```python
from build123d import *

# Parameters (mm, degrees)
V_BLOCK_BODY_100_DEPTH    = 100
CENTRAL_CHANNEL_SKETCH_W  = 36
CENTRAL_CHANNEL_SKETCH_H  = 12
CENTRAL_CHANNEL_CUT_DEPTH = 166
SQUARE_POCKET_18X18_REACH = 179.739
SQUARE_START              = -32
SQUARE_POCKET_SKETCH_W    = 88
SQUARE_POCKET_SKETCH_H    = 60
ANGLED_NOTCH_CUT_REACH    = 131.46


with BuildPart() as part:
    # V-Block Profile Sketch → V-Block Body 100 (new body)
    with BuildSketch(Plane.XY):
        Polygon((-30, 43), (0, 13), (30, 43), (62, 43), (62, -43), (-62, -43), (-62, 43), align=None)
    extrude(amount=V_BLOCK_BODY_100_DEPTH)

    # Central Channel Sketch → Central Channel Cut (cut, through all)
    with BuildSketch(Plane.ZY.offset(62)):
        with Locations((50, -37)):
            Rectangle(CENTRAL_CHANNEL_SKETCH_W, CENTRAL_CHANNEL_SKETCH_H)
        Polygon((40, 43), (100, -11), (100, 43), align=None)
    extrude(amount=-CENTRAL_CHANNEL_CUT_DEPTH, mode=Mode.SUBTRACT)

    # Square Pocket 18x18: up to this face of the body (flat: up to its plane)
    square_pocket_18x18_end = Plane(part.part.faces().sort_by_distance((-46, 43, 20))[0])
    # Square Pocket Sketch → Square Pocket 18x18 (cut, up to the picked face)
    with BuildSketch(Plane.XZ.offset(43).offset(SQUARE_START), mode=Mode.PRIVATE) as square_pocket_18x18_sk1:
        with Locations((0, 70)):
            Rectangle(SQUARE_POCKET_SKETCH_W, SQUARE_POCKET_SKETCH_H)
    square_pocket_18x18_tool1 = split(extrude(square_pocket_18x18_sk1.sketch, amount=-SQUARE_POCKET_18X18_REACH, mode=Mode.PRIVATE), bisect_by=square_pocket_18x18_end, keep=Keep.BOTH, mode=Mode.PRIVATE)
    add(square_pocket_18x18_tool1.solids().sort_by(Axis((0, -11, 70), (0, 1, 0)))[0], mode=Mode.SUBTRACT)

    # Angled Notch Sketch → Angled Notch Cut (cut, up to next)
    with BuildSketch(Plane(origin=(0, -11, 0), x_dir=(1, 0, 0), z_dir=(0, 1, 0)), mode=Mode.PRIVATE) as angled_notch_cut_sk1:
        Polygon((-18, -100), (0, -82), (18, -100), align=None)
    angled_notch_cut_tool1 = extrude(angled_notch_cut_sk1.sketch, amount=-ANGLED_NOTCH_CUT_REACH, mode=Mode.PRIVATE) & part.part
    add(angled_notch_cut_tool1.solids().sort_by_distance((0, -11, 94))[0], mode=Mode.SUBTRACT)


solid = part.part
```
Design review of the part built by this model. Coordinates are the model's own, in mm. A direction names the side the tool comes from. Give positions to 0.01 mm unless a question says otherwise; leave off trailing zeros. Order: outer loops, then holes, each group sorted by start corner. A loop starts at its lowest first (then second) coordinate and runs counter-clockwise, first axis right, second up. Notation, with made-up numbers: M -38,-25.5 L -31,-25.5 A25 cw -31,5.5 Z; hole C 47,80.5 d6. An arc over 180 degrees is marked long. One line per question, with ' | ' between items. Start each with the question number.
Q1. For pin 1 Ø4 at (x, z) = (-4, 63.5) entering from +Y, flat-tipped, find the tip position at first contact; note if it passes through.
Q2. We need section A-A (y = -29.5). Write out the cut boundary in (x, z), plus the area to 3 significant figures.
Q3. For L1, parallel to X at y = 16.5, z = 52; L2, parallel to Z at x = -16, y = -7; L3, parallel to X at y = 21, z = 23.5, list the stretches that pass through material, from the lowest coordinate up. Write a range as [from, to].
Q4. The part is to be moulded in two halves that separate along Z. For faces 4 (the face through (-1, -37, 32)), 5 (the face through (-9, -27, 91)), 6 (the face through (44, 10, 63)), say which applies: +Z half, -Z half, draft (parallel to the pull), parting line (faces both ways), or undercut.
Q5. We need section B-B (z = 23). Write out the cut boundary in (x, y), plus the area to 3 significant figures.
Q6. We need section D-D (y = 18.5). Write out the cut boundary in (x, z), plus the area to 3 significant figures.
Q7. We need section C-C (x = -15.5). Write out the cut boundary in (y, z), plus the area to 3 significant figures.
Q8. Machinability: for faces 1 (the face through (15, 28, 20)), 2 (the face through (-44, 10, 63)), 3 (the face through (9, -27, 91)), which of the approach directions +Z, -Z, +X, -X, +Y, -Y give a long, thin tool a straight path to every point of the face, cutting with its end or side? Answer none if there is none.
Returned:
1) pin 1: y = -11
2) outline: M -62,0 L 62,0 L 62,100 L 18,100 L 0,82 L -18,100 L -62,100 Z | area: 12,100 mm2
3) L1: [-62, -44], [44, 62] | L2: [0, 40] | L3: [-62, -8], [8, 62]
4) face 4: undercut | face 5: +Z half | face 6: draft
5) outline: M -62,-43 L 62,-43 L 62,43 L 30,43 L 0,13 L -30,43 L -62,43 Z | area: 9,760 mm2
6) outline: M -62,0 L -5.5,0 L -5.5,40 L -44,40 L -44,67.22 L -62,67.22 Z; M 5.5,0 L 62,0 L 62,67.22 L 44,67.22 L 44,40 L 5.5,40 Z | area: 5,500 mm2
7) outline: M -43,0 L 28.5,0 L 28.5,40 L -11,40 L -11,97.5 L -43,97.5 L -43,68 L -31,68 L -31,32 L -43,32 Z | area: 4,270 mm2
8) face 1: +Z, -Z, +Y | face 2: +Z, +Y | face 3: +Z, +Y, -Y
